Geometry: see drawing. Coordinates: mm, zero at the bounding-box minimum. A direction names the side the tool comes from. Coordinates: 2 decimals unless noted, no trailing zeros. Loops run counter-clockwise (first coordinate to the right, second up) from the corner with the lowest first, then second, coordinate; pieces in that order, holes last. Notation, with made-up numbers: (80.25, -36.75) - (103.25, -36.75) arc R9 ccw to (103.25, -24.75) - close; hole circle Ø7 at (24.25, 33). An arc over 180 degrees is marked (long way). Use one line per item in the form item = value.
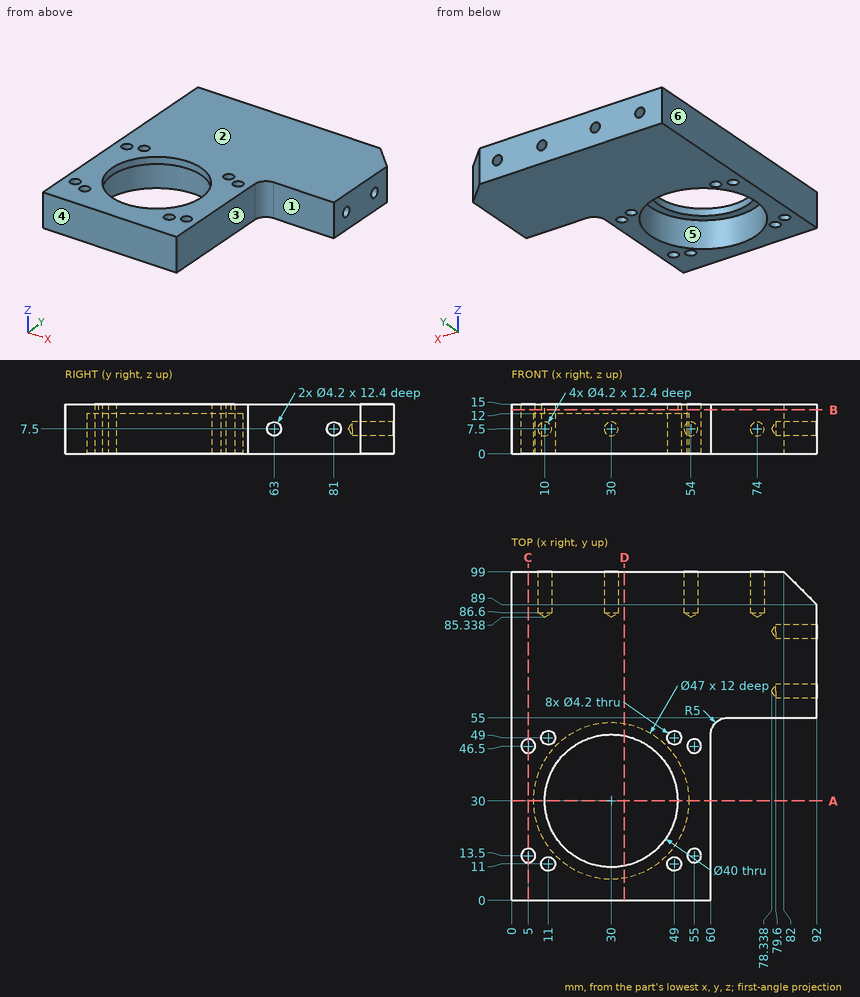
Q1. First-contact query: P1, Ø12, axis at x = 16.5, y = 23, coming from the -Z side; P2, Ø4, axis at x = 54, z = 7.5, coming from the +Y side; P3, Ø6, axis at x = 52.5, z = 11, coming from the -Y side; P4, Ø2.5, axis at x = 55, y = 13.5, coming from the +Z side. Flat tips, straight axial feed; report the tip coordinate or a pass-through.
Check values:
P1 = 12
P2 = 86.54
P3 = 0
P4 = through
Q2. Cut plane B-B, the plane z = 13.25. Give the number of separate pieces and of enclosed holes in the cut face, then the cut area to 3 significant figures.
Check values:
separate_pieces = 1
enclosed_holes = 9
area = 5,940 mm²
Q3. Ray query, line 1 along Y through (x, z) = (5, 10.25); line 2 along X through (y, z) = (48, 7.5); line 3 along Y through (x, z) = (49, 8.75). Return the intervals inside material, ascending. Write a range as [from, to].
Check values:
line_1 = [0, 11.4], [15.6, 44.4], [48.6, 99]
line_2 = [0, 3.53], [6.47, 9.15], [12.85, 14.89], [45.11, 47.15], [50.85, 53.53], [56.47, 60]
line_3 = [0, 8.9], [13.1, 16.17], [43.83, 46.9], [51.1, 99]
Q4. Cut plane D-D, the plane x = 34. Return loops of the section in (y, z), then the cut area to 3 significant figures.
Check values:
outline = (0, 0) - (6.84, 0) - (6.84, 12) - (10.4, 12) - (10.4, 15) - (0, 15) - close; (49.6, 12) - (53.16, 12) - (53.16, 0) - (99, 0) - (99, 15) - (49.6, 15) - close
area = 812 mm²
Q5. Cut plane A-A, the plane y = 30. Return loops of the section in (x, z), then the cut area to 3 significant figures.
Check values:
outline = (0, 0) - (6.5, 0) - (6.5, 12) - (10, 12) - (10, 15) - (0, 15) - close; (50, 12) - (53.5, 12) - (53.5, 0) - (60, 0) - (60, 15) - (50, 15) - close
area = 216 mm²
Q6. Cut plane C-C, the plane x = 5. Return loops of the section in (y, z), then the cut area to 3 significant figures.
Check values:
outline = (0, 0) - (11.4, 0) - (11.4, 15) - (0, 15) - close; (15.6, 0) - (44.4, 0) - (44.4, 15) - (15.6, 15) - close; (48.6, 0) - (99, 0) - (99, 15) - (48.6, 15) - close
area = 1,360 mm²
Q7. Pull-direction query (X, two-part tool) for the marked faces 3, 4, 5 and 6; classes: pulls with the +X half, pulls with the -X half, needs draft (parallel to the pull), parting line crosses it, or undercut.
Check values:
face_3 = pulls with the +X half
face_4 = needs draft
face_5 = undercut
face_6 = pulls with the -X half
Q8. Set-up query: the marked faces 1 and 2. Return all of +Z, -Z, +X, -X, +Y, -Y with unobstructed straight access to the full face (end or side cutting, diameter ignored); none if empty.
Check values:
face_1 = +Z, -Z, +X, -Y
face_2 = +Z, +X, -X, +Y, -Y
